The model under review builds one solid part; all positions refer to its coordinate system, in mm. A direction names the side the tool comes from. Coordinates: 2 decimals unless noted, no trailing zeros. Order: outer loops, then holes, each group sorted by start corner. A loop starts at its lowest first (then second) coordinate and runs counter-clockwise, first axis right, second up.
from build123d import *

# Parameters (mm, degrees)
BASE_PROFILE_13MM_DEPTH    = 13
UPRIGHT_BLOCK_82MM_DEPTH   = 82
RECTANGULAR_CUT_SKETCH_W   = 54
RECTANGULAR_CUT_SKETCH_H   = 50
RECTANGULAR_CUT_20MM_DEPTH = 20
POCKET_CUT_SKETCH_W        = 13
POCKET_CUT_SKETCH_H        = 32
POCKET_CUT_13MM_DEPTH      = 13
SLOT_CUT_14MM_DEPTH        = 13
MOUNTING_FLANGE_6MM_DEPTH  = 13
FLANGE_HOLES_SKETCH_R      = 6
FLANGE_HOLES_2X_12_DEPTH   = 13


with BuildPart() as part:
    # Base Profile Sketch → Base Profile 13mm (new body)
    with BuildSketch(Plane.XY):
        with BuildLine():
            Line((0, 0), (100, 0))
            Line((100, 0), (100, 82))
            Line((100, 82), (68, 82))
            Line((68, 82), (68, 38))
            ThreePointArc((68, 38), (66.242640687, 33.757359313), (62, 32))
            Line((62, 32), (0, 32))
            Line((0, 32), (0, 0))
        make_face()
    extrude(amount=BASE_PROFILE_13MM_DEPTH)

    # Upright Block Sketch → Upright Block 82mm (add)
    with BuildSketch(Plane.XZ):
        with BuildLine():
            Line((19, 0), (0, 0))
            Line((0, 0), (0, -54))
            Line((0, -54), (13, -54))
            Line((13, -54), (13, -6))
            ThreePointArc((13, -6), (14.757359313, -1.757359313), (19, 0))
        make_face()
        with BuildLine():
            Line((100, 0), (81, 0))
            ThreePointArc((81, 0), (85.242640687, -1.757359313), (87, -6))
            Line((87, -6), (87, -26))
            Line((87, -26), (100, -26))
            Line((100, -26), (100, 0))
        make_face()
    extrude(amount=-UPRIGHT_BLOCK_82MM_DEPTH)

    # Rectangular Cut Sketch → Rectangular Cut 20mm (cut)
    with BuildSketch(Plane.ZY):
        with Locations((-27, 57)):
            Rectangle(RECTANGULAR_CUT_SKETCH_W, RECTANGULAR_CUT_SKETCH_H)
    extrude(amount=-RECTANGULAR_CUT_20MM_DEPTH, mode=Mode.SUBTRACT)

    # Pocket Cut Sketch → Pocket Cut 13mm (cut)
    with BuildSketch(Plane(origin=(0, 0, -54), x_dir=(-1, 0, 0), z_dir=(0, 0, -1))):
        with Locations((-6.5, 16)):
            Rectangle(POCKET_CUT_SKETCH_W, POCKET_CUT_SKETCH_H)
    extrude(amount=-POCKET_CUT_13MM_DEPTH, mode=Mode.SUBTRACT)

    # Slot Cut Sketch → Slot Cut 14mm (cut)
    with BuildSketch(Plane.ZY):
        with BuildLine():
            Line((-41, 9), (-26, 9))
            ThreePointArc((-26, 9), (-19, 16), (-26, 23))
            Line((-26, 23), (-41, 23))
            Line((-41, 23), (-41, 9))
        make_face()
    extrude(amount=-SLOT_CUT_14MM_DEPTH, mode=Mode.SUBTRACT)

    # Mounting Flange Sketch → Mounting Flange 6mm (add)
    with BuildSketch(Plane(origin=(0, 0, -26), x_dir=(-1, 0, 0), z_dir=(0, 0, -1))):
        with BuildLine():
            Line((-100, 82), (-176, 82))
            Line((-176, 82), (-176, 50))
            Line((-176, 50), (-106, 50))
            ThreePointArc((-106, 50), (-101.757359313, 48.242640687), (-100, 44))
            Line((-100, 44), (-100, 82))
        make_face()
    extrude(amount=-MOUNTING_FLANGE_6MM_DEPTH)

    # Flange Holes Sketch → Flange Holes 2xØ12 (cut)
    with BuildSketch(Plane.XY.offset(-13)):
        with Locations((116, 66.156876682)):
            Circle(FLANGE_HOLES_SKETCH_R)
        with Locations((160, 66.156876682)):
            Circle(FLANGE_HOLES_SKETCH_R)
    extrude(amount=-FLANGE_HOLES_2X_12_DEPTH, mode=Mode.SUBTRACT)


solid = part.part
(1) Consider section D-D (z = 10). Give the boundary of the cut face in (x, y), then the cut area to 3 significant figures.
(2) Wall thickness on line 1 (Y direction, x = 160, z = -20.75); line 2 (X direction, y = 16.5, z = -13); line 3 (Z direction, x = 79, y = 63): over which ranges is each line inside the solid? List them lowest first.
(3) Consider section B-B (z = -32). Give the boundary of the cut face in (x, y), then the cut area to 3 significant figures.
(4) Tool access review of faces 1 (the face through (87, 40, -16)), 2 (the face through (6, 23, -33)), 3 (the face through (6, 16, -19)), 4 (the face through (139, 63, -13)), 5 (the face through (18, 32, 4)): name each direction out of +Z, -Z, +X, -X, +Y, -Y from which nothing blocks a thin tool from reaching the whole face with its end or side.
(5) Consider section C-C (y = 55). Give the boundary of the cut face in (x, z).
(6) Consider section A-A (x = 116). Give the boundary of the cut face in (y, z).
(7) The part is to be moulded in two halves that separate along X. For faces 6 (the face through (68, 60, 6)), 7 (the face through (100, 40, -2)), 8 (the face through (56, 23, 0)), say which applies: +X half, -X half, draft (parallel to the pull), parting line (faces both ways), or undercut.
(8) Insertion check: pin 1 Ø10 at (x, z) = (62.5, -1.5) entering from +Y; pin 2 Ø4 at (y, z) = (21.5, -2) entering from -X; pin 3 Ø6 at (y, z) = (35.5, -18) entering from -X; pin 4 Ø6.5 at (x, z) = (7, -31.5) entering from +Y. Each pin has a flat end and moves straight along its axis. Give the tip position at first contact, or say it passes through.
Findings:
1. outline: (0, 0) - (100, 0) - (100, 82) - (68, 82) - (68, 38) arc R6 cw to (62, 32) - (0, 32) - close
1. area: 4,810 mm2
2. line 1: y = 50 to 60.16, 72.16 to 82
2. line 2: x = 0 to 13, 87 to 100
2. line 3: z = 0 to 13
3. outline: (0, 0) - (13, 0) - (13, 9) - (0, 9) - close; (0, 23) - (13, 23) - (13, 32) - (0, 32) - close
3. area: 234 mm2
4. face 1: -Z, +Y, -Y
4. face 2: -Z, +X, -X
4. face 3: -Z, -X
4. face 4: +Z, +X, +Y, -Y
4. face 5: +Z, -Z, -X, +Y
5. outline: (68, 0) - (81, 0) arc R6 cw to (87, -6) - (87, -26) - (176, -26) - (176, -13) - (100, -13) - (100, 13) - (68, 13) - close
6. outline: (50, -26) - (60.16, -26) - (60.16, -13) - (50, -13) - close; (72.16, -26) - (82, -26) - (82, -13) - (72.16, -13) - close
7. face 6: -X half
7. face 7: +X half
7. face 8: undercut
8. pin 1: stops at y = 35.13
8. pin 2: stops at x = 0
8. pin 3: stops at x = 87
8. pin 4: stops at y = 32
